Input: part model. Units: mm. Frame: model coordinates. A direction names the side the tool comes from. Coordinates: 2 decimals unless noted, no trailing zeros. Write each loop counter-clockwise with the first axis right and the second up, starting at its lowest first coordinate (ties: lowest second). Pieces come first, ordered by that corner, then holes. Notation, with made-up numbers: (73.5, 41.25) - (114.5, 41.25) arc R13 ccw to (114.5, 51.25) - close; hole circle Ø9 at (28, -27). An arc over 180 degrees is marked (long way). Put each result on its own line as item: value. Start each with the question number.
1. Pin query (flat end, axial travel): pin 1 (1 mm diameter, centred on y = -2.5, z = -53, fed in from -X); pin 2 (3 mm diameter, centred on y = 12, z = -60.5, fed in from -X); pin 3 (1 mm diameter, centred on x = 16.5, z = -154.5, fed in from +Y). Return the tip coordinate at first contact, or that it passes through.
2. Cut plane C-C, the plane z = 53.5. Return loops of the section in (x, y), and give its area (3 significant figures).
3. Cut plane A-A, the plane y = 0. Return loops of the section in (x, z), and give its area (3 significant figures).
4. Line query: line 1 (Z direction, x = 7, y = 20); line 2 (Z direction, x = 12, y = 2); line 3 (Y direction, x = 1.5, z = -234). Output: solid intervals per line, ascending.
5. Access query for faces 1 (the cylindrical face through (4.336, -19.524, -251.756)), 2 (the flat face through (0, 0, -346)). Directions: +Z, -Z, +X, -X, +Y, -Y. A direction counts if a zero-diameter tool reaches every point of the face in a straight line with its end or side. Return the directions, or none.
from build123d import *

# Parameters (mm, degrees)
EXTRUDE_1_DEPTH      = 100
EXTRUDE_1_DEPTH_BACK = 346
SKETCH_1_R           = 25
SKETCH_2_R           = 25
SKETCH_2_R_2         = 20
CUT_EXTRUDE_1_DEPTH  = 109
SKETCH_3_R           = 25
SKETCH_3_R_2         = 12
CUT_EXTRUDE_2_DEPTH  = 40
CHAMFER_1_SIZE       = 1


with BuildPart() as part:
    # 草图1 → 凸台-拉伸1 (new, two sides: drawn at the far end of the back side and taken through both)
    with BuildSketch(Plane.XY.offset(-EXTRUDE_1_DEPTH_BACK)):
        Circle(SKETCH_1_R)
    extrude(amount=EXTRUDE_1_DEPTH + EXTRUDE_1_DEPTH_BACK)

    # 草图2 → 切除-拉伸1 (cut)
    with BuildSketch(Plane(origin=(0, 0, -306), x_dir=(-1, 0, 0), z_dir=(0, 0, -1))):
        with Locations(Location((0, 0, 0), (0, 0, 180))):
            Circle(SKETCH_2_R)
        Circle(SKETCH_2_R_2, mode=Mode.SUBTRACT)
    extrude(amount=-CUT_EXTRUDE_1_DEPTH, mode=Mode.SUBTRACT)

    # 草图3 → 切除-拉伸2 (cut)
    with BuildSketch(Plane(origin=(0, 0, -346), x_dir=(-1, 0, 0), z_dir=(0, 0, -1))):
        with Locations(Location((0, 0, 0), (0, 0, 180))):
            Circle(SKETCH_3_R)
        Circle(SKETCH_3_R_2, mode=Mode.SUBTRACT)
    extrude(amount=-CUT_EXTRUDE_2_DEPTH, mode=Mode.SUBTRACT)

    # 倒角1
    chamfer_1_edges = [part.edges().sort_by_distance(p)[0] for p in [
        (20, 0, -306),
        (12, 0, -346),
        (-25, 0, -197),
    ]]
    chamfer(chamfer_1_edges, length=CHAMFER_1_SIZE)


solid = part.part
Report:
1. pin 1: stops at x = -24.92
1. pin 2: stops at x = -22.69
1. pin 3: stops at y = 19.21
2. outline: circle Ø50 at (0, 0)
2. area: 1,960 mm^2
3. outline: (-25, -196) - (-24, -197) - (-20, -197) - (-20, -305) - (-19, -306) - (-12, -306) - (-12, -345) - (-11, -346) - (11, -346) - (12, -345) - (12, -306) - (19, -306) - (20, -305) - (20, -197) - (24, -197) - (25, -196) - (25, 100) - (-25, 100) - close
3. area: 20,200 mm^2
4. line 1: z = -197 to 100
4. line 2: z = -306 to 100
4. line 3: y = -19.94 to 19.94
5. face 1: -Z
5. face 2: -Z, +X, -X, +Y, -Y
